Check sheet for the modelled part. Datum: model origin and axes. Units: mm. A direction names the side the tool comes from. Round coordinates to 2 decimals unless told otherwise and drop trailing zeros. Loops run counter-clockwise (first coordinate to the right, second up) from the corner with the lowest first, then second, coordinate; pieces in that order, holes last. Notation, with made-up numbers: (-26.75, 84.5) - (19.25, 84.5) arc R28 ccw to (19.25, 122.5) - close; hole circle Ø2 at (2.5, 17.5). An arc over 180 degrees is marked (long way). Answer in a Markdown table with one row per item. Add a question column.
(1) Cross-section at C-C on x = -45.5. Enter the section's corners in (y, z), then the cut area to 3 significant figures.
(2) Cross-section at A-A on y = 23. Enter the section's corners in (x, z).
(3) Cross-section at D-D on z = 50. Enter the section's corners in (x, y).
(4) Cross-section at B-B on y = 86.5. Enter the section's corners in (x, z), then the cut area to 3 significant figures.
(5) Thickness scan on line 1 along X through (y, z) = (84.5, 0); line 2 along Y through (x, z) = (-25, 53); line 3 along X through (y, z) = (72, 0) (3 decimals). Record the ranges inside material, lowest first.
(6) Gauge pin test, flat ends, axial feed: pin 1 (22.5 mm diameter, centred on x = 26.5, y = 86, fed in from +Z); pin 2 (1.5 mm diameter, centred on x = -57.5, z = 12, fed in from +Y); pin 3 (1.5 mm diameter, centred on x = 18, z = 2.5, fed in from -Y); pin 4 (7 mm diameter, centred on x = -28, y = 27, fed in from -Z). Record the tip position at first contact, or that the pin passes through.
(7) Mould release check, pull along Z, two halves, no side actions. Record for faces 5 (the cylindrical face through (28.92, 85.12, 0.07)), 6 (the cylindrical face through (13.52, 49.3, -14.74)), 7 (the flat face through (-66, 8, 60)): +Z half, -Z half, draft (parallel to the pull), parting line (faces both ways), or undercut.
(8) Access from +Z, -Z, +X, -X, +Y, -Y to the whole of each face (thin tool, end or side, straight path). Record for faces 1 (the cylindrical face through (-35.23, 31.39, 0.04)), 2 (the flat face through (-63, 76, -4)), 3 (the flat face through (-60.446, 42.17, 2.558)), 4 (the flat face through (-72.62, 38.25, 18.88)).
from build123d import *

# Parameters (mm, degrees)
COLUMN_PROFILE_SKETCH_R   = 20
COLUMN_BOSS_DEPTH         = 100
BASE_ARM_PLATE_DEPTH      = 20
COLUMN_BORE_30_D          = 30
COLUMN_BORE_30_DEPTH      = 42
COLUMN_BORE_30_TIP        = 9.012909285
HOOK_GUIDE_BLOCK_SKETCH_R = 10
HOOK_GUIDE_BLOCK_DEPTH    = 10
HOOK_SLOT_CUT_DEPTH       = 138.652199764
HOOK_RECESS_SKETCH_R      = 20
HOOK_RECESS_20_DEPTH      = 8
CLAMP_LUG_SKETCH_W        = 21.478013603
CLAMP_LUG_SKETCH_H        = 10
CLAMP_LUG_DEPTH           = 40
CLAMP_LUG_FILLET_R10_R    = 10
CLAMP_HOLES_SKETCH_R      = 5
CLAMP_HOLES_2X_10_DEPTH   = 40
EYE_LUG_DEPTH             = 3


with BuildPart() as part:
    # Column Profile Sketch → Column Boss (new body)
    with BuildSketch(Plane(origin=(0, 0, 0), x_dir=(1, 0, 0), z_dir=(0, 1, 0))):
        with Locations(Location((0, 0, 0), (0, 0, 270))):
            Circle(COLUMN_PROFILE_SKETCH_R)
    extrude(amount=COLUMN_BOSS_DEPTH)

    # Base Arm Profile Sketch → Base Arm Plate (add)
    with BuildSketch(Plane(origin=(0, 0, 0), x_dir=(1, 0, 0), z_dir=(0, 1, 0))):
        with BuildLine():
            Line((0, 20), (-62, 20))
            Line((-62, 20), (-78.41, -20))
            Line((-78.41, -20), (-78.41, -50))
            ThreePointArc((-78.41, -50), (-52.871711259, -79.666363657), (-19.737124491, -58.82418325))
            ThreePointArc((-19.737124491, -58.82418325), (-7.771853725, -35.023523327), (11.344775373, -16.471067717))
            ThreePointArc((11.344775373, -16.471067717), (-19.097399749, -5.9404817), (0, 20))
        make_face()
    extrude(amount=BASE_ARM_PLATE_DEPTH)

    # Column Bore Ø30
    with Locations(Plane.ZX.offset(100)):
        with Locations((0, 0)):
            Hole(COLUMN_BORE_30_D / 2, depth=COLUMN_BORE_30_DEPTH)
            with Locations((0, 0, -(COLUMN_BORE_30_DEPTH + COLUMN_BORE_30_TIP / 2))):  # 118° drill point
                Cone(0, COLUMN_BORE_30_D / 2, COLUMN_BORE_30_TIP, mode=Mode.SUBTRACT)

    # Hook Guide Block Sketch → Hook Guide Block (add)
    with BuildSketch(Plane(origin=(-60.091325676, 0, -24.652466359), x_dir=(-0.3795512800466907, 0, 0.9251707009060105), z_dir=(-0.9251707009060105, 0, -0.3795512800466907))):
        with BuildLine():
            Line((5.028765345, 20), (5.028765345, 66))
            ThreePointArc((5.028765345, 66), (7.957697533, 73.071067812), (15.028765345, 76))
            Line((15.028765345, 76), (25.028765345, 76))
            ThreePointArc((25.028765345, 76), (39.170900969, 70.142135624), (45.028765345, 56))
            Line((45.028765345, 56), (45.028765345, 20))
            Line((45.028765345, 20), (5.028765345, 20))
        make_face()
        with Locations((25.028765345, 56)):
            Circle(HOOK_GUIDE_BLOCK_SKETCH_R, mode=Mode.SUBTRACT)
    extrude(amount=-HOOK_GUIDE_BLOCK_DEPTH)

    # Hook Slot Sketch → Hook Slot Cut (cut, through all)
    with BuildSketch(Plane(origin=(0, 20, 0), x_dir=(1, 0, 0), z_dir=(0, 1, 0))):
        with BuildLine():
            Line((-48.41, -40), (-78.41, -40))
            Line((-78.41, -40), (-78.41, -60))
            Line((-78.41, -60), (-48.41, -60))
            ThreePointArc((-48.41, -60), (-38.41, -50), (-48.41, -40))
        make_face()
    extrude(amount=-HOOK_SLOT_CUT_DEPTH, mode=Mode.SUBTRACT)

    # Hook Recess Sketch → Hook Recess Ø20 (cut)
    with BuildSketch(Plane(origin=(0, 20, 0), x_dir=(1, 0, 0), z_dir=(0, 1, 0))):
        with Locations((-48.41, -50)):
            Circle(HOOK_RECESS_SKETCH_R)
    extrude(amount=-HOOK_RECESS_20_DEPTH, mode=Mode.SUBTRACT)

    # Clamp Lug Sketch → Clamp Lug (add)
    with BuildSketch(Plane(origin=(0, 100, 0), x_dir=(1, 0, 0), z_dir=(0, 1, 0))):
        with Locations((29.260993199, 0)):
            Rectangle(CLAMP_LUG_SKETCH_W, CLAMP_LUG_SKETCH_H)
    extrude(amount=-CLAMP_LUG_DEPTH)

    # Clamp Lug Fillet R10
    clamp_lug_fillet_r10_edges = [part.edges().sort_by_distance(p)[0] for p in [
        (40, 60, 0),
        (40, 100, 0),
    ]]
    fillet(clamp_lug_fillet_r10_edges, radius=CLAMP_LUG_FILLET_R10_R)

    # Clamp Holes Sketch → Clamp Holes 2xØ10 (cut)
    with BuildSketch(Plane.XY.offset(5)):
        with Locations((30, 90)):
            Circle(CLAMP_HOLES_SKETCH_R)
        with Locations((30, 70)):
            Circle(CLAMP_HOLES_SKETCH_R)
    extrude(amount=-CLAMP_HOLES_2X_10_DEPTH, mode=Mode.SUBTRACT)

    # Eye Lug Sketch → Eye Lug (add, symmetric)
    with BuildSketch(Plane.XY):
        with BuildLine():
            Line((-44, 20), (-44, 26))
            ThreePointArc((-44, 26), (-35.12324798, 31.496493808), (-29.780131863, 40.466403549))
            ThreePointArc((-29.780131863, 40.466403549), (-27.972203076, 43.020697561), (-25, 44))
            Line((-25, 44), (-20, 44))
            Line((-20, 44), (-17, 44))
            Line((-17, 44), (-17, 20))
            Line((-17, 20), (-44, 20))
        make_face()
    extrude(amount=EYE_LUG_DEPTH, both=True)


solid = part.part
Answers:
| question | item | result |
|---|---|---|
| 1 | outline | (0, -20) - (20, -20) - (20, 30.21) - (12, 30.21) - (12, 40.43) - (0, 40.43) - close; (0, 59.57) - (12, 59.57) - (12, 69.79) - (20, 69.79) - (20, 79.86) - (0, 79.86) - close |
| 1 | area | 1,450 mm^2 |
| 2 | outline | (-77.18, 17.01) - (-62, -20) - (-52.75, -16.2) - (-67.93, 20.8) - close; (-44, -3) - (-19.77, -3) arc R20 ccw (long way) to (-19.77, 3) - (-44, 3) - close |
| 3 | outline | (-38.41, 0) - (-16.44, 0) - (-16.44, 20) - (-28.41, 20) - (-28.41, 12) - (-38.41, 12) - close |
| 4 | outline | (19.36, -5) - (26.43, -5) - (26.43, 5) - (19.36, 5) arc R20 ccw (long way) to start; (33.57, -5) - (40, -5) - (40, 5) - (33.57, 5) - close; hole circle Ø30 at (0, 0) |
| 4 | area | 680 mm^2 |
| 5 | line 1 | x = -20 to -15, 15 to 40 |
| 5 | line 2 | y = 0 to 20 |
| 5 | line 3 | x = -70.205 to -59.396, -20 to -15, 15 to 25.417, 34.583 to 40 |
| 6 | pin 1 | stops at z = 12.94 |
| 6 | pin 2 | stops at y = 20 |
| 6 | pin 3 | stops at y = 0 |
| 6 | pin 4 | stops at z = -3 |
| 7 | face 5 | draft |
| 7 | face 6 | parting line |
| 7 | face 7 | undercut |
| 8 | face 1 | +Z, -Z, +Y |
| 8 | face 2 | +Z, -Z, -X, +Y |
| 8 | face 3 | +Z, +Y |
| 8 | face 4 | +Z, -X, +Y |
